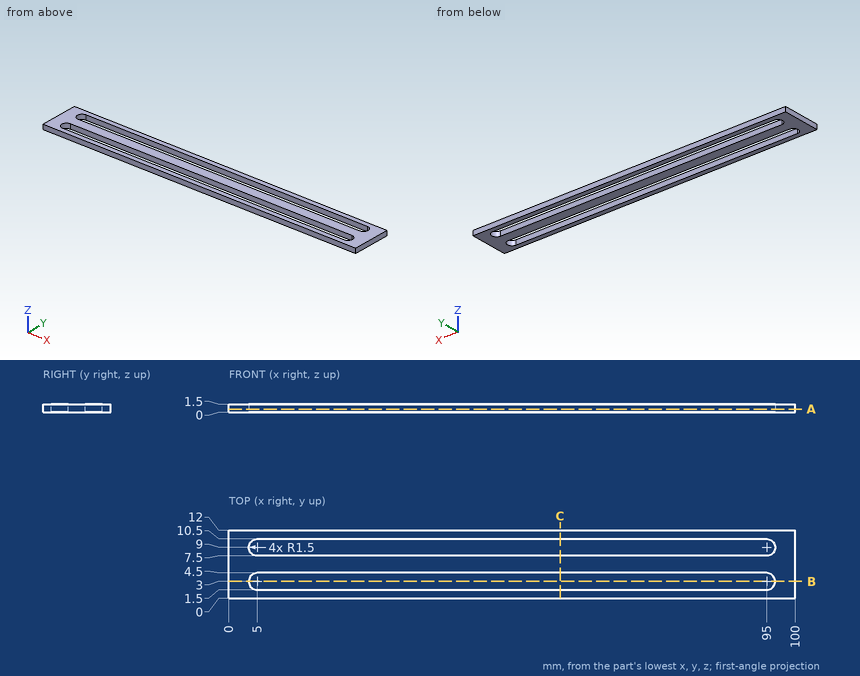
Input: dimensioned drawing with shaded views. Units: mm. Origin: part minimum x, y, z. Coordinates: 2 decimals unless noted, no trailing zeros. Write each loop counter-clockwise with the first axis right and the second up, starting at its lowest first coordinate (ties: lowest second). Pieces come first, ordered by that corner, then holes. Notation, with made-up numbers: (-26.5, -14) -> (-1.5, -14) arc R16 cw to (-1.5, 9) -> close; hole circle Ø4 at (36, 26). An arc over 180 degrees is marked (long way). Return JSON: item names as keys, results as strings. Group by question number.
1) Section query B-B, the plane y = 3. Return loops of the section in (x, z), plus the area to 3 significant figures.
2) Ray query, line 1 along Y through (x, z) = (59, 0.95); line 2 along X through (y, z) = (3, 0.35); line 3 along X through (y, z) = (2, 1.05). Return the intervals inside material, ascending.
3) Section query A-A, the plane z = 0.6. Return loops of the section in (x, y).
4) Section query C-C, the plane x = 58.5. Return loops of the section in (y, z), plus the area to 3 significant figures.
From the geometry:
{
 "1": {"outline": "(0, 0) -> (3.5, 0) -> (3.5, 1.5) -> (0, 1.5) -> close; (96.5, 0) -> (100, 0) -> (100, 1.5) -> (96.5, 1.5) -> close", "area": "10.5 mm²"},
 "2": {"line 1": "0 to 1.5, 4.5 to 7.5, 10.5 to 12", "line 2": "0 to 3.5, 96.5 to 100", "line 3": "0 to 3.88, 96.12 to 100"},
 "3": {"outline": "(0, 0) -> (100, 0) -> (100, 12) -> (0, 12) -> close; hole (5, 1.5) -> (95, 1.5) arc R1.5 ccw to (95, 4.5) -> (5, 4.5) arc R1.5 ccw to start; hole (5, 7.5) -> (95, 7.5) arc R1.5 ccw to (95, 10.5) -> (5, 10.5) arc R1.5 ccw to start"},
 "4": {"outline": "(0, 0) -> (1.5, 0) -> (1.5, 1.5) -> (0, 1.5) -> close; (4.5, 0) -> (7.5, 0) -> (7.5, 1.5) -> (4.5, 1.5) -> close; (10.5, 0) -> (12, 0) -> (12, 1.5) -> (10.5, 1.5) -> close", "area": "9.00 mm²"}
}
